from build123d import *

# Parameters (mm, degrees)
SKETCH1_R           = 7.5
BOSS_EXTRUDE1_DEPTH = 138
SKETCH2_R           = 5.5
BOSS_EXTRUDE2_DEPTH = 20
SKETCH3_R           = 5.5
BOSS_EXTRUDE3_DEPTH = 45
CHAMFER1_SIZE       = 1
BOSS_EXTRUDE4_START = 46
SKETCH4_R           = 5.5
BOSS_EXTRUDE4_DEPTH = 46
CHAMFER2_SIZE       = 1


with BuildPart() as part:
    # Sketch1 → Boss-Extrude1 (new body)
    with BuildSketch(Plane.XY):
        Circle(SKETCH1_R)
    extrude(amount=BOSS_EXTRUDE1_DEPTH)

    # Sketch2 → Boss-Extrude2 (add)
    with BuildSketch(Plane.XY.offset(138)):
        Circle(SKETCH2_R)
    extrude(amount=BOSS_EXTRUDE2_DEPTH)

    # Sketch3 → Boss-Extrude3 (add)
    with BuildSketch(Plane.XY.offset(158)):
        Circle(SKETCH3_R)
    extrude(amount=BOSS_EXTRUDE3_DEPTH)

    # Chamfer1
    chamfer1_edges = [part.edges().sort_by_distance(p)[0] for p in [
        (-7.5, 0, 0),
        (-7.5, 0, 138),
        (-5.5, 0, 203),
    ]]
    chamfer(chamfer1_edges, length=CHAMFER1_SIZE)

    # Sketch4 → Boss-Extrude4 (add)
    with BuildSketch(Plane(origin=(0, 0, 0), x_dir=(-1, 0, 0), z_dir=(0, 0, -1)).offset(BOSS_EXTRUDE4_START)):
        with Locations(Location((0, 0, 0), (0, 0, 180))):
            Circle(SKETCH4_R)
    extrude(amount=-BOSS_EXTRUDE4_DEPTH)

    # Chamfer2
    chamfer2_edges = [part.edges().sort_by_distance(p)[0] for p in [
        (-5.5, 0, -46),
    ]]
    chamfer(chamfer2_edges, length=CHAMFER2_SIZE)


solid = part.part
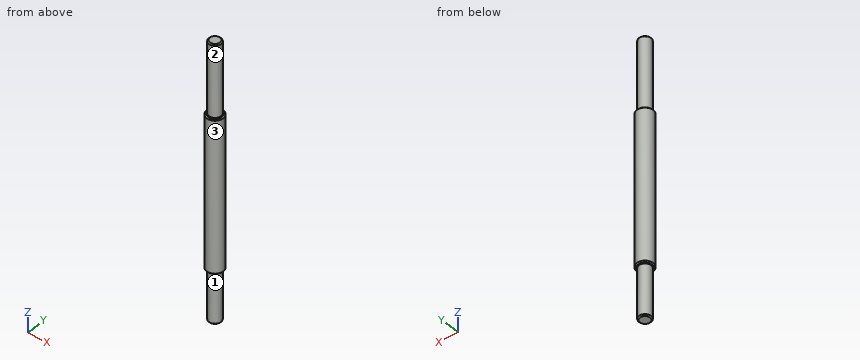
Verification items for the finished model (mm, model axes). Face numbers are marked on the shaded views. A direction names the side the tool comes from. Coordinates: 2 decimals unless noted, no trailing zeros. Loops run counter-clockwise (first coordinate to the right, second up) from the corner with the lowest first, then second, coordinate; pieces in that order, holes last. Notation, with made-up numbers: M 38,8 L 69,8 A10 ccw 69,12 Z; hole C 10.25,-2.5 d10. An arc over 180 degrees is marked long. One line per item, written item: value.
1. Section check D-D on z = 162. Record the cut outline in (x, y), plus the area to 3 significant figures.
Answers follow:
outline: C 0,0 d11
area: 95.0 mm^2
2. Set-up check for the marked faces 1, 2 and 3: record each of +Z, -Z, +X, -X, +Y, -Y from which the full face is reachable in a straight line by a thin tool's end or side.
Answers follow:
face 1: -Z
face 2: +Z
face 3: +Z, -Z
3. Material ranges on line 1 along X through (y, z) = (6, 7); line 2 along X through (y, z) = (3.75, 16); line 3 along Z through (x, y) = (6, -2), recorded low to high. Write a range as from..to.
Answers follow:
line 1: -4.5..4.5
line 2: -6.5..6.5
line 3: 0..138
4. Section check C-C on z = 49.5. Record the cut outline in (x, y), plus the area to 3 significant figures.
Answers follow:
outline: C 0,0 d15
area: 177 mm^2
5. Gauge pin test, flat ends, axial feed: P1, Ø3, axis at y = -4, z = 45.5, coming from the +X side; P2, Ø8, axis at x = 6, z = 111, coming from the +Y side; P3, Ø3, axis at x = 0.5, y = -4.5, coming from the +Z side; P4, Ø4, axis at x = 5, z = 119, coming from the +Y side. Record the tip position at first contact, or that the pin passes through.
Answers follow:
P1: x = 7.07
P2: y = 7.23
P3: z = 203
P4: y = 6.87
6. Section check A-A on x = 0. Record the cut outline in (y, z).
Answers follow:
outline: M -7.5,1 L -6.5,0 L -5.5,0 L -5.5,-45 L -4.5,-46 L 4.5,-46 L 5.5,-45 L 5.5,0 L 6.5,0 L 7.5,1 L 7.5,137 L 6.5,138 L 5.5,138 L 5.5,202 L 4.5,203 L -4.5,203 L -5.5,202 L -5.5,138 L -6.5,138 L -7.5,137 Z
